Verification items for the finished model (mm, model axes). Face numbers are marked on the shaded views. A direction names the side the tool comes from. Round coordinates to 2 decimals unless told otherwise and drop trailing zeros. Write each loop counter-clockwise with the first axis right and the second up, starting at its lowest first coordinate (ties: lowest second). Pieces come first, ordered by that corner, then holes. Notation, with made-up numbers: M 9.25,17.5 L 26.25,17.5 A16 ccw 26.25,23.5 Z; hole C -10,-4 d9. An arc over 180 degrees is marked long. Use a Markdown table: item, result. Add a question column.
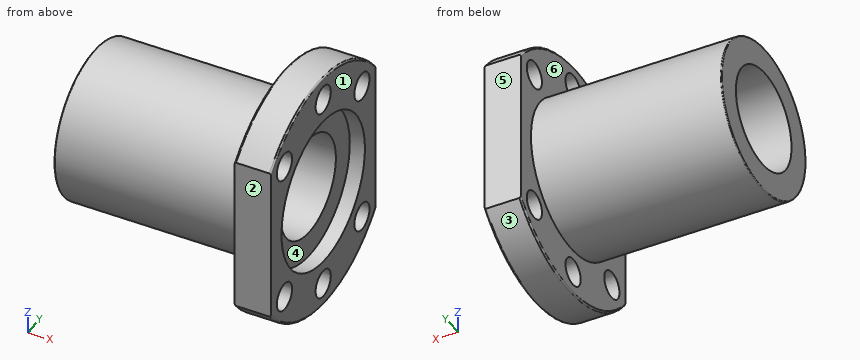
from build123d import *

# Parameters (mm, degrees)
EXTRUDE_1_DEPTH               = 11.999999998
SKETCH_2_W                    = 63.000000153
SKETCH_2_H                    = 24.999999254
HOLE_WIZARD_9_0_9_1_D         = 9
HOLE_WIZARD_M30_1_D           = 32.999998421
HOLE_WIZARD_M30_1_CBORE_D     = 49.499997436
HOLE_WIZARD_M30_1_CBORE_DEPTH = 5
FILLET_1_R                    = 0.3
FILLET_2_R                    = 0.5


with BuildPart() as part:
    # 草图1 → 凸台-拉伸1 (new body)
    with BuildSketch(Plane(origin=(-19.893035878, 0, 0), x_dir=(0, 0, -1), z_dir=(1, 0, 0))):
        with BuildLine():
            Line((25.278447364, 30.999999739), (-25.278447364, 30.999999739))
            ThreePointArc((-25.278447364, 30.999999739), (-39.999998764, -2.61e-07), (-25.278447364, -31.000000261))
            Line((-25.278447364, -31.000000261), (25.278447364, -31.000000261))
            ThreePointArc((25.278447364, -31.000000261), (39.999998764, -2.61e-07), (25.278447364, 30.999999739))
        make_face()
    extrude(amount=-EXTRUDE_1_DEPTH)

    # 草图2 → 旋转1 (revolve)
    with BuildSketch(Plane.XY, mode=Mode.PRIVATE) as revolve_1_sk:
        with Locations((-63.393035954, 12.499998381)):
            Rectangle(SKETCH_2_W, SKETCH_2_H)
    revolve(revolve_1_sk.sketch.rotate(Axis((-94.89303603, -1.246e-06, 0), (1, 0, 0)), 270), axis=Axis((-94.89303603, -1.246e-06, 0), (1, 0, 0)))

    # Ø9.0 (9) 直径孔1 (through all)
    with Locations(Plane.ZY.offset(31.893035877)):
        with Locations((22.981, 22.980999581), (22.981, -22.981000419), (-22.981, -22.981000419), (-22.981, 22.980999581), (32.5, -4.19e-07), (-32.5, -4.19e-07)):
            Hole(HOLE_WIZARD_9_0_9_1_D / 2)

    # M30 六角头螺栓的柱形沉头孔1 (through all)
    with Locations(Plane(origin=(-19.893035878, 0, 0), x_dir=(0, 0, -1), z_dir=(1, 0, 0))):
        with Locations((0, -2.61e-07)):
            CounterBoreHole(HOLE_WIZARD_M30_1_D / 2, HOLE_WIZARD_M30_1_CBORE_D / 2, HOLE_WIZARD_M30_1_CBORE_DEPTH)

    # 圆角1
    fillet_1_edges = [part.edges().sort_by_distance(p)[0] for p in [
        (-94.89303603, -1.246e-06, 24.999999255),
    ]]
    fillet(fillet_1_edges, radius=FILLET_1_R)

    # 圆角2
    fillet_2_edges = [part.edges().sort_by_distance(p)[0] for p in [
        (-31.893035877, -2.61e-07, 39.999998764),
        (-31.893035877, -2.61e-07, -39.999998764),
        (-19.893035878, -2.61e-07, 39.999998764),
        (-19.893035878, -2.61e-07, -39.999998764),
    ]]
    fillet(fillet_2_edges, radius=FILLET_2_R)


solid = part.part
1. Cross-section at D-D on z = -21. Count the separate pieces of the cut face and the enclosed holes in it, plus the area to 3 significant figures.
2. Release check for a two-part mould opening along Y. For the marked faces 1, 2, 3 and 4 record: +Y half, -Y half, draft (parallel to the pull), parting line (faces both ways), or undercut.
3. Scan lines: line 1 along Z through (x, y) = (-24, 0); line 2 along Z through (x, y) = (-25, 0); line 3 along Z through (x, y) = (-27.5, -24.5). Record each from-to range of solid material in increasing order. Write a range as from..to.
4. Cross-section at B-B on x = -29. Enter the section's corners in (y, z), plus the area to 3 significant figures.
5. Depth check by flat-ended pin: pin 1 Ø4 at (x, z) = (-62.5, -6) entering from -Y; pin 2 Ø10.5 at (y, z) = (0, 32.5) entering from +X; pin 3 Ø14.5 at (y, z) = (-22.981, 22.981) entering from -X; pin 4 Ø1.5 at (x, z) = (-36.5, -17) entering from +Y. Enter the tip coordinate at first touch or a pass-through.
6. Access from +Z, -Z, +X, -X, +Y, -Y to the whole of each face (thin tool, end or side, straight path). Record for the marked faces 5 and 6.
7. Cross-section at A-A on z = 0. Enter the section's corners in (x, y), plus the area to 3 significant figures.
8. Cross-section at C-C on x = -77. Enter the section's corners in (y, z), plus the area to 3 significant figures.
Answer:
| question | item | result |
|---|---|---|
| 1 | separate pieces | 3 |
| 1 | enclosed holes | 0 |
| 1 | area | 2,130 mm^2 |
| 2 | face 1 | draft |
| 2 | face 2 | -Y half |
| 2 | face 3 | parting line |
| 2 | face 4 | undercut |
| 3 | line 1 | z = -40..-37, -28..-24.75, 24.75..28, 37..40 |
| 3 | line 2 | z = -40..-37, -28..-16.5, 16.5..28, 37..40 |
| 3 | line 3 | z = -31.62..-27.22, -18.75..18.75, 27.22..31.62 |
| 4 | outline | M -31,-25.28 A40 ccw 31,-25.28 L 31,25.28 A40 ccw -31,25.28 Z; hole C -22.98,-22.98 d9; hole C -22.98,22.98 d9; hole C 0,0 d33; hole C 0,-32.5 d9; hole C 0,32.5 d9; hole C 22.98,-22.98 d9; hole C 22.98,22.98 d9 |
| 4 | area | 3,170 mm^2 |
| 5 | pin 1 | stops at y = -24.68 |
| 5 | pin 2 | stops at x = -19.89 |
| 5 | pin 3 | stops at x = -31.89 |
| 5 | pin 4 | stops at y = 19 |
| 6 | face 5 | +Z, -Z, +X, -X, +Y |
| 6 | face 6 | -X |
| 7 | outline | M -94.89,-24.7 A0.3 ccw -94.59,-25 L -31.89,-25 L -31.89,-31 L -19.89,-31 L -19.89,-24.75 L -24.89,-24.75 L -24.89,-16.5 L -94.89,-16.5 Z; M -94.89,16.5 L -24.89,16.5 L -24.89,24.75 L -19.89,24.75 L -19.89,31 L -31.89,31 L -31.89,25 L -94.59,25 A0.3 ccw -94.89,24.7 Z |
| 7 | area | 1,340 mm^2 |
| 8 | outline | C 0,0 d50; hole C 0,0 d33 |
| 8 | area | 1,110 mm^2 |
